For this review, take the finished solid that the model builds, in its own axes (mm). Face numbers are marked on the shaded views. A direction names the side the tool comes from. Coordinates: 2 decimals unless noted, no trailing zeros. Write each loop counter-clockwise with the first axis right and the second up, starting at its lowest first coordinate (ties: lowest second). Pieces come first, ordered by that corner, then holes. Notation, with made-up numbers: (45.25, 88.25) -> (96.25, 88.25) arc R14 ccw to (96.25, 113.25) -> close; hole circle Ø8 at (-30, 22.5). An arc over 180 degrees is marked (long way). One line per item, written item: value. Start each with the question number.
1) For probe 1 along X at (y, z) = (33.5, 1); probe 2 along X at (y, z) = (-14, -27); probe 3 along Z at (x, y) = (173.5, 1.5), list the stretches that pass through material, from the lowest coordinate up. Write a range as from..to.
2) Add section A-A (x = 60.5). State the section outline as (y, z) points.
3) Machinability: for the marked faces 1, 2 and 3, which of the approach directions +Z, -Z, +X, -X, +Y, -Y give a long, thin tool a straight path to every point of the face, cutting with its end or side? Answer none if there is none.
4) Add section B-B (x = 178.5). State the section outline as (y, z) points, and give its area (3 significant figures).
5) For pin 1 Ø6 at (x, z) = (59, -1.5) entering from -Y; pin 2 Ø5 at (x, y) = (40, 22.5) entering from -Z; pin 3 Ø8 at (y, z) = (-31.5, 30) entering from -X, all flat-tipped, find the tip position at first contact; note any pin that passes through.
from build123d import *

# Parameters (mm, degrees)
CHAMFER1_SIZE      = 1
CHAMFER2_SIZE      = 1
FILLET1_R          = 0.5
CHAMFER3_SIZE      = 1
CHAMFER4_SIZE      = 1
FILLET2_R          = 0.5
CUT_EXTRUDE1_START = 19.5
CUT_EXTRUDE1_DEPTH = 20
CUT_EXTRUDE2_START = 27.5
CUT_EXTRUDE2_DEPTH = 20


with BuildPart() as part:
    # Sketch1 → Revolve3 (revolve)
    with BuildSketch(Plane.XY, mode=Mode.PRIVATE) as revolve3_sk:
        Polygon((0, 0), (0, 25), (96, 25), (96, 28.5), (148, 28.5), (148, 30), (199, 30), (199, 35), (262, 35), (262, 40), (270, 40), (270, 34.5), (278, 34.5), (278, 30), (312, 30), (312, 0), align=None)
    revolve(revolve3_sk.sketch.rotate(Axis((0, 0, 0), (1, 0, 0)), 90), axis=Axis((0, 0, 0), (1, 0, 0)))

    # Chamfer1
    chamfer1_edges = [part.edges().sort_by_distance(p)[0] for p in [
        (0, 0, -25),
    ]]
    chamfer(chamfer1_edges, length=CHAMFER1_SIZE)

    # Chamfer2
    chamfer2_edges = [part.edges().sort_by_distance(p)[0] for p in [
        (312, 0, -30),
    ]]
    chamfer(chamfer2_edges, length=CHAMFER2_SIZE)

    # Fillet1
    fillet1_edges = [part.edges().sort_by_distance(p)[0] for p in [
        (148, 0, -28.5),
        (96, 0, -25),
    ]]
    fillet(fillet1_edges, radius=FILLET1_R)

    # Chamfer3
    chamfer3_edges = [part.edges().sort_by_distance(p)[0] for p in [
        (199, 0, -35),
    ]]
    chamfer(chamfer3_edges, length=CHAMFER3_SIZE)

    # Chamfer4
    chamfer4_edges = [part.edges().sort_by_distance(p)[0] for p in [
        (96, 0, -28.5),
    ]]
    chamfer(chamfer4_edges, length=CHAMFER4_SIZE)

    # Fillet2
    fillet2_edges = [part.edges().sort_by_distance(p)[0] for p in [
        (199, 0, -30),
    ]]
    fillet(fillet2_edges, radius=FILLET2_R)

    # Sketch2 → Cut-Extrude1 (cut)
    with BuildSketch(Plane(origin=(0, 0, 0), x_dir=(1, 0, 0), z_dir=(0, 1, 0)).offset(CUT_EXTRUDE1_START)):
        with BuildLine():
            Line((20, 7), (76, 7))
            ThreePointArc((76, 7), (83, 0), (76, -7))
            Line((76, -7), (20, -7))
            ThreePointArc((20, -7), (13, 0), (20, 7))
        make_face()
    extrude(amount=CUT_EXTRUDE1_DEPTH, mode=Mode.SUBTRACT)

    # Sketch3 → Cut-Extrude2 (cut)
    with BuildSketch(Plane(origin=(0, 0, 0), x_dir=(1, 0, 0), z_dir=(0, 1, 0)).offset(CUT_EXTRUDE2_START)):
        with BuildLine():
            Line((212.5, 10), (248.5, 10))
            ThreePointArc((248.5, 10), (258.5, 0), (248.5, -10))
            Line((248.5, -10), (212.5, -10))
            ThreePointArc((212.5, -10), (202.5, 0), (212.5, 10))
        make_face()
    extrude(amount=CUT_EXTRUDE2_DEPTH, mode=Mode.SUBTRACT)


solid = part.part
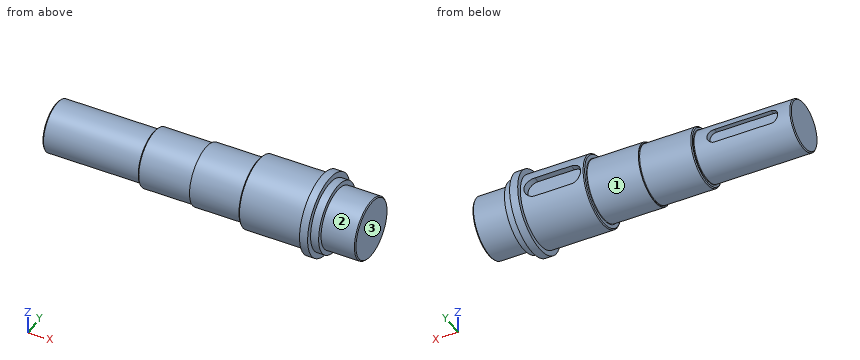
Numbers:
1. probe 1: 199..202.55, 258.45..278
1. probe 2: 198.99..278
1. probe 3: -29.96..29.96
2. outline: (19.5, -7) -> (19.5, 7) -> (24, 7) arc R25 ccw (long way) to (24, -7) -> close
3. face 1: -X
3. face 2: +X
3. face 3: +Z, -Z, +X, +Y, -Y
4. outline: circle Ø60 at (0, 0)
4. area: 2,830 mm²
5. pin 1: y = -25
5. pin 2: z = -15
5. pin 3: x = 262
